The model under review builds one solid part; all positions refer to its coordinate system, in mm. A direction names the side the tool comes from. Round coordinates to 2 decimals unless told otherwise and drop trailing zeros. Order: outer loops, then holes, each group sorted by start corner. A loop starts at its lowest first (then second) coordinate and runs counter-clockwise, first axis right, second up. Notation, with made-up numbers: M -12,8 L 16,8 A23 ccw 16,34 Z; hole C 72.25,-28.5 d7. An arc over 180 degrees is marked long. Answer as CSV lines item,"result". Start each with the question number.
from build123d import *

# Parameters (mm, degrees)
FORK_PROFILE_SKETCH_R   = 25
FORK_BASE_BODY_DEPTH    = 35
SKETCH2_3_R             = 17.5
HUB_BOSS_DEPTH          = 51
HUB_BORE_DEPTH          = 55
FORK_ARMS_DEPTH         = 17.5
PIN_HOLE_SKETCH_R       = 6
CROSS_PIN_HOLE_12_DEPTH = 140


with BuildPart() as part:
    # Fork Profile Sketch → Fork Base Body (new, symmetric)
    with BuildSketch(Plane(origin=(0, 0, 0), x_dir=(1, 0, 0), z_dir=(0, 1, 0))):
        with Locations(Location((0, 0, 0), (0, 0, 270))):
            Circle(FORK_PROFILE_SKETCH_R)
    extrude(amount=FORK_BASE_BODY_DEPTH, both=True)

    # Sketch2_3 → Hub Boss (add)
    with BuildSketch(Plane(origin=(0, 0, 0), x_dir=(1, 0, 0), z_dir=(0, 1, 0))):
        with Locations(Location((0, 0, 0), (0, 0, 270))):
            Circle(SKETCH2_3_R)
    extrude(amount=HUB_BOSS_DEPTH)

    # Sketch2_4 → Hub Bore (cut, symmetric)
    with BuildSketch(Plane(origin=(0, 0, 0), x_dir=(1, 0, 0), z_dir=(0, 1, 0))):
        with BuildLine():
            Line((9.946400687, -1.033979392), (0, -1.717163069))
            Line((0, -1.717163069), (-9.946400687, -1.033979392))
            ThreePointArc((-9.946400687, -1.033979392), (0, -10), (9.946400687, -1.033979392))
        make_face()
        with BuildLine():
            Line((-9.946400687, -1.033979392), (0, -1.717163069))
            Line((0, -1.717163069), (9.946400687, -1.033979392))
            ThreePointArc((9.946400687, -1.033979392), (9.986591182, -0.517683849), (10, 0))
            ThreePointArc((10, 0), (-0.517683849, 9.986591182), (-9.946400687, -1.033979392))
        make_face()
        with BuildLine():
            Line((9.946400687, -1.033979392), (0, -1.717163069))
            Line((0, -1.717163069), (-9.946400687, -1.033979392))
            ThreePointArc((-9.946400687, -1.033979392), (0, -10), (9.946400687, -1.033979392))
        make_face()
        with BuildLine():
            Line((-9.946400687, -1.033979392), (0, -1.717163069))
            Line((0, -1.717163069), (9.946400687, -1.033979392))
            ThreePointArc((9.946400687, -1.033979392), (9.986591182, -0.517683849), (10, 0))
            ThreePointArc((10, 0), (-0.517683849, 9.986591182), (-9.946400687, -1.033979392))
        make_face()
    extrude(amount=HUB_BORE_DEPTH, both=True, mode=Mode.SUBTRACT)

    # Sketch2_5 → Fork Arms (add, symmetric)
    with BuildSketch(Plane(origin=(0, 0, 0), x_dir=(1, 0, 0), z_dir=(0, 1, 0))):
        with BuildLine():
            ThreePointArc((25, 0), (0, -25), (-25, 0))
            Line((-25, 0), (-25, -65))
            Line((-25, -65), (-40, -65))
            Line((-40, -65), (-40, -107))
            Line((-40, -107), (-30, -107))
            Line((-30, -107), (-30, -75))
            Line((-30, -75), (-15, -75))
            Line((-15, -75), (-15, -35))
            Line((-15, -35), (15, -35))
            Line((15, -35), (15, -52.523875455))
            Line((15, -52.523875455), (15, -75))
            Line((15, -75), (30, -75))
            Line((30, -75), (30, -107))
            Line((30, -107), (40, -107))
            Line((40, -107), (40, -65))
            Line((40, -65), (25, -65))
            Line((25, -65), (25, 0))
        make_face()
    extrude(amount=FORK_ARMS_DEPTH, both=True)

    # Pin Hole Sketch → Cross Pin Hole _12 (cut)
    with BuildSketch(Plane(origin=(40, 0, 0), x_dir=(0, 0, -1), z_dir=(1, 0, 0))):
        with Locations((-88, 0)):
            Circle(PIN_HOLE_SKETCH_R)
    extrude(amount=-CROSS_PIN_HOLE_12_DEPTH, mode=Mode.SUBTRACT)


solid = part.part
Item 1: Wall thickness on probe 1 along X at (y, z) = (-10, 54); probe 2 along Y at (x, z) = (-33, 88); probe 3 along X at (y, z) = (0.5, 69.5): over which ranges is each line inside the solid? List them lowest first. Write a range as [from, to].
Item 2: Consider section A-A (z = 67). State the section outline as (x, y) points, and give its area (3 significant figures).
Item 3: The part is to be moulded in two halves that separate along X. For faces 4 (the flat face through (-5, 35, -17)), 5 (the flat face through (-23, 0, 75)), 6 (the cylindrical face through (1.099, 0.49, -24.976)), 7 (the flat face through (-40, 0, 81)), say which applies: +X half, -X half, draft (parallel to the pull), parting line (faces both ways), or undercut.
Item 4: Consider section D-D (z = 88). State the section outline as (x, y) points.
Item 5: Consider section B-B (y = 0). State the section outline as (x, z) points, and give its area (3 significant figures).
Item 6: Tool access review of faces 1 (the cylindrical face through (-10.648, 42.888, -13.887)), 2 (the flat face through (-32, 0, 65)), 3 (the flat face through (0, 0, 35)): name each direction out of +Z, -Z, +X, -X, +Y, -Y from which nothing blocks a thin tool from reaching the whole face with its end or side.
Item 7: Consider section C-C (x = 0). State the section outline as (y, z) points.
Item 8: For pin 1 (2 mm diameter, centred on x = -4.5, y = -3.5, fed in from +Z); pin 2 (12 mm diameter, centred on x = -32, y = 2, fed in from -Z); pin 3 (4 mm diameter, centred on y = -14.5, z = 51.5, fed in from -X); pin 4 (9.5 mm diameter, centred on y = 0, z = 88, fed in from -X), all flat-tipped, find the tip position at first contact; note any pin that passes through.
Reported:
1,probe 1,"x = [-25, -15], [15, 25]"
1,probe 2,"y = [-17.5, -6], [6, 17.5]"
1,probe 3,"x = [-40, -15], [15, 40]"
2,outline,"M -40,-17.5 L -15,-17.5 L -15,17.5 L -40,17.5 Z; M 15,-17.5 L 40,-17.5 L 40,17.5 L 15,17.5 Z"
2,area,"1,750 mm²"
3,face 4,"draft"
3,face 5,"undercut"
3,face 6,"parting line"
3,face 7,"-X half"
4,outline,"M -40,-17.5 L -30,-17.5 L -30,-6 L -40,-6 Z; M -40,6 L -30,6 L -30,17.5 L -40,17.5 Z; M 30,-17.5 L 40,-17.5 L 40,-6 L 30,-6 Z; M 30,6 L 40,6 L 40,17.5 L 30,17.5 Z"
5,outline,"M -40,65 L -25,65 L -25,0 A25 ccw 25,0 L 25,65 L 40,65 L 40,82 L 30,82 L 30,75 L 15,75 L 15,35 L -15,35 L -15,75 L -30,75 L -30,82 L -40,82 Z; M -40,94 L -30,94 L -30,107 L -40,107 Z; M 30,94 L 40,94 L 40,107 L 30,107 Z; hole C 0,0 d20"
5,area,"3,920 mm²"
6,face 1,"+Y"
6,face 2,"-Z, -X, +Y, -Y"
6,face 3,"+Z, +Y, -Y"
7,outline,"M -35,-25 L 35,-25 L 35,-17.5 L 51,-17.5 L 51,-10 L -35,-10 Z; M -35,10 L 51,10 L 51,17.5 L 35,17.5 L 35,25 L 17.5,25 L 17.5,35 L -17.5,35 L -17.5,25 L -35,25 Z"
8,pin 1,"stops at z = 35"
8,pin 2,"stops at z = 65"
8,pin 3,"stops at x = -25"
8,pin 4,"passes through"
